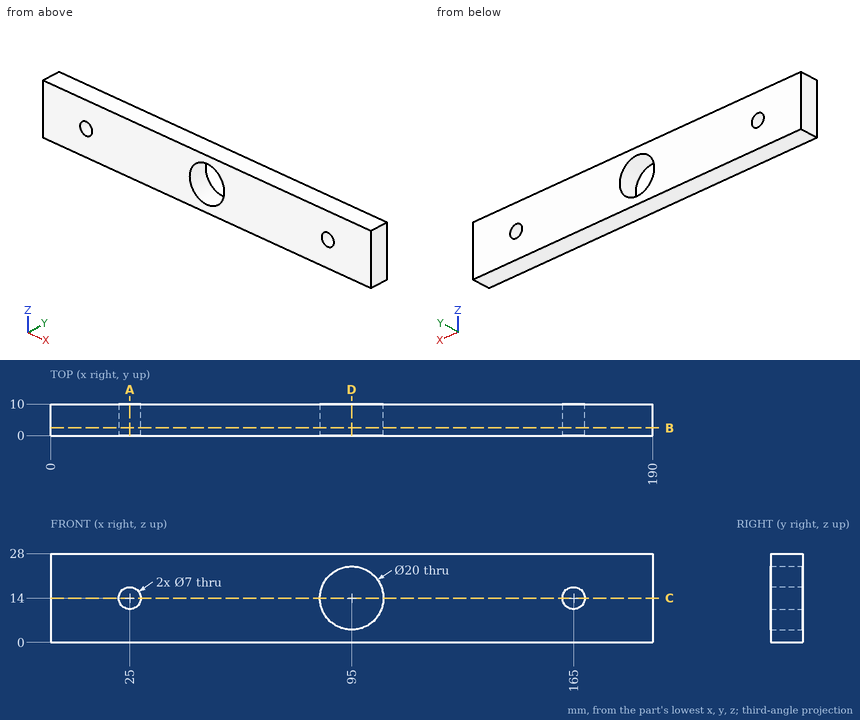
Study the drawing (mm; zero at the part's minimum x, y, z) and answer. Round coordinates to 2 decimals unless told otherwise and drop trailing zeros. Write each loop counter-clockwise with the first axis right and the second up, starting at its lowest first coordinate (ties: lowest second). Pieces come first, ordered by that corner, then holes.
1) A cutting plane is placed at A-A on x = 25. Determine the outline of the cut face in (y, z), and give its area (3 significant figures).
2) A cutting plane is placed at C-C on z = 14. Determine the outline of the cut face in (x, y).
3) A cutting plane is placed at D-D on x = 95. Determine the outline of the cut face in (y, z), and give its area (3 significant figures).
4) A cutting plane is placed at B-B on y = 2.5. Determine the outline of the cut face in (x, z).
5) Consider probe 1 along Z at (x, y) = (165, 4.5); probe 2 along Z at (x, y) = (95, 2.5); probe 3 along X at (y, z) = (3.75, 15.75). Determine where each line is inside the solid, lowest interval first.
Entries:
1. outline: (0, 0) - (10, 0) - (10, 10.5) - (0, 10.5) - close; (0, 17.5) - (10, 17.5) - (10, 28) - (0, 28) - close
1. area: 210 mm2
2. outline: (0, 0) - (21.5, 0) - (21.5, 10) - (0, 10) - close; (28.5, 0) - (85, 0) - (85, 10) - (28.5, 10) - close; (105, 0) - (161.5, 0) - (161.5, 10) - (105, 10) - close; (168.5, 0) - (190, 0) - (190, 10) - (168.5, 10) - close
3. outline: (0, 0) - (10, 0) - (10, 4) - (0, 4) - close; (0, 24) - (10, 24) - (10, 28) - (0, 28) - close
3. area: 80.0 mm2
4. outline: (0, 0) - (190, 0) - (190, 28) - (0, 28) - close; hole circle Ø7 at (25, 14); hole circle Ø20 at (95, 14); hole circle Ø7 at (165, 14)
5. probe 1: z = 0 to 10.5, 17.5 to 28
5. probe 2: z = 0 to 4, 24 to 28
5. probe 3: x = 0 to 21.97, 28.03 to 85.15, 104.85 to 161.97, 168.03 to 190
